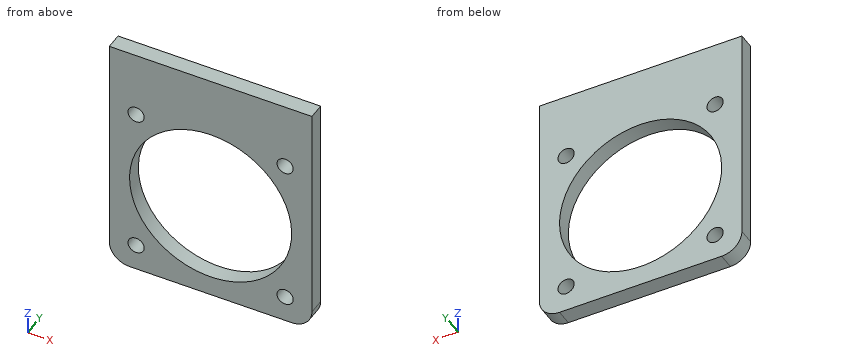
```python
from build123d import *

# Parameters (mm, degrees)
SKETCH1_W                = 100
SKETCH1_H                = 120
BOSS_EXTRUDE1_DEPTH      = 8
FILLET1_R                = 10
CUT_EXTRUDE1_REACH       = 80.511
SKETCH2_R                = 40
F_8_0_8_DIAMETER_HOLE1_D = 8
CIRPATTERN1_COUNT        = 4


with BuildPart() as part:
    # Sketch1 → Boss-Extrude1 (new body)
    with BuildSketch(Plane(origin=(0, 0, 0), x_dir=(1, 0, 0), z_dir=(0, 1, 0))):
        Rectangle(SKETCH1_W, SKETCH1_H)
    extrude(amount=BOSS_EXTRUDE1_DEPTH)

    # Fillet1
    fillet1_edges = [part.edges().sort_by_distance(p)[0] for p in [
        (-50, 4, -60),
        (50, 4, -60),
    ]]
    fillet(fillet1_edges, radius=FILLET1_R)

    # Sketch2 → Cut-Extrude1 (cut, up to next)
    with BuildSketch(Plane(origin=(0, 8, 0), x_dir=(1, 0, 0), z_dir=(0, 1, 0)), mode=Mode.PRIVATE) as cut_extrude1_sk1:
        with Locations(Location((0, 10, 0), (0, 0, 270))):
            Circle(SKETCH2_R)
    cut_extrude1_tool1 = extrude(cut_extrude1_sk1.sketch, amount=-CUT_EXTRUDE1_REACH, mode=Mode.PRIVATE) & part.part
    add(cut_extrude1_tool1.solids().sort_by_distance((0, 8, -10))[0], mode=Mode.SUBTRACT)

    # Ø8.0 (8) Diameter Hole1 (through all)
    with Locations(Plane(origin=(0, 8, 0), x_dir=(1, 0, 0), z_dir=(0, 1, 0))):
        with Locations((-36.769552622, 46.769552622)):
            f_8_0_8_diameter_hole1 = Hole(F_8_0_8_DIAMETER_HOLE1_D / 2)

    # CirPattern1: Ø8.0 (8) Diameter Hole1 ×4 about axis
    cirpattern1_axis = Axis((0, 0, -10), (0, 1, 0))
    for i in range(1, CIRPATTERN1_COUNT):
        add(f_8_0_8_diameter_hole1.rotate(cirpattern1_axis, i * 360 / CIRPATTERN1_COUNT), mode=Mode.SUBTRACT)


solid = part.part
```
Design review of the part built by this model. Coordinates are the model's own, in mm. Coordinates: 2 decimals unless noted, no trailing zeros. Write each loop counter-clockwise with the first axis right and the second up, starting at its lowest first coordinate (ties: lowest second). Pieces come first, ordered by that corner, then holes. Notation, with made-up numbers: M -28,-3 L 8,-3 A28 cw 8,31 Z; hole C 18.5,83.5 d4. An arc over 180 degrees is marked long. Answer as a JSON object with one key per item and string values.
Item 1: Add section A-A, the plane z = -10. Give the boundary of the cut face in (x, y).
Outcome:
{"outline": "M -50,0 L -40,0 L -40,8 L -50,8 Z; M 40,0 L 50,0 L 50,8 L 40,8 Z"}
Item 2: Add section B-B, the plane x = 0. Give the boundary of the cut face in (y, z).
Outcome:
{"outline": "M 0,-60 L 8,-60 L 8,-50 L 0,-50 Z; M 0,30 L 8,30 L 8,60 L 0,60 Z"}
Item 3: Wall thickness on probe 1 along X at (y, z) = (3.25, -43.5); probe 2 along X at (y, z) = (4.5, -45); probe 3 along Z at (x, y) = (-36, 7.25): over which ranges is each line inside the solid? List them lowest first.
Outcome:
{"probe 1": "-50 to -39.07, -34.47 to -21.86, 21.86 to 34.47, 39.07 to 50", "probe 2": "-50 to -40.36, -33.18 to -19.36, 19.36 to 33.18, 40.36 to 50", "probe 3": "-60 to -50.69, -42.84 to -27.44, 7.44 to 22.84, 30.69 to 60"}
Item 4: Add section C-C, the plane y = 4.25. Give the boundary of the cut face in (x, z), and give its area (3 significant figures).
Outcome:
{"outline": "M -50,-50 A10 ccw -40,-60 L 40,-60 A10 ccw 50,-50 L 50,60 L -50,60 Z; hole C -36.77,-46.77 d8; hole C -36.77,26.77 d8; hole C 0,-10 d80; hole C 36.77,-46.77 d8; hole C 36.77,26.77 d8", "area": "6,730 mm²"}
